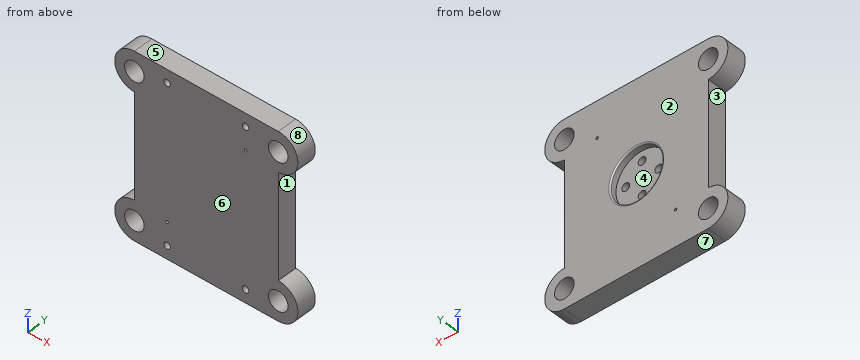
```python
from build123d import *

# Parameters (mm, degrees)
SKETCH1_R                                        = 15
BOSS_EXTRUDE1_DEPTH                              = 30
CBORE_FOR_M8_PAN_HEAD_MACHINE_SCREW1_D           = 9
CBORE_FOR_M8_PAN_HEAD_MACHINE_SCREW1_CBORE_D     = 18
CBORE_FOR_M8_PAN_HEAD_MACHINE_SCREW1_CBORE_DEPTH = 6
SKETCH_1_R                                       = 2
CUT_EXTRUDE1_DEPTH                               = 201.249843945
SKETCH_3_R                                       = 5
CUT_EXTRUDE3_DEPTH                               = 20
SKETCH_4_R                                       = 40
CUT_EXTRUDE4_DEPTH                               = 10
FILLET1_R                                        = 2
SKETCH5_R                                        = 6
CUT_EXTRUDE7_DEPTH                               = 15


with BuildPart() as part:
    # Sketch1 → Boss-Extrude1 (new body)
    with BuildSketch(Plane(origin=(0, 0, 0), x_dir=(1, 0, 0), z_dir=(0, 1, 0))):
        with BuildLine():
            Line((-110, -140), (80, -140))
            Line((80, -140), (80, 140))
            Line((80, 140), (-110, 140))
            ThreePointArc((-110, 140), (-140, 110), (-110, 80))
            Line((-110, 80), (-110, -80))
            ThreePointArc((-110, -80), (-140, -110), (-110, -140))
        make_face()
        with Locations(Location((-110, 110, 0), (0, 0, 270))):
            Circle(SKETCH1_R, mode=Mode.SUBTRACT)
        with Locations(Location((-110, -110, 0), (0, 0, 270))):
            Circle(SKETCH1_R, mode=Mode.SUBTRACT)
    boss_extrude1 = extrude(amount=BOSS_EXTRUDE1_DEPTH)

    # CBORE for M8 Pan Head Machine Screw1 (through all)
    with Locations(Plane(origin=(0, 30, 0), x_dir=(1, 0, 0), z_dir=(0, 1, 0))):
        with Locations((60, 120), (-60, 120), (-60, -120), (60, -120)):
            CounterBoreHole(CBORE_FOR_M8_PAN_HEAD_MACHINE_SCREW1_D / 2, CBORE_FOR_M8_PAN_HEAD_MACHINE_SCREW1_CBORE_D / 2, CBORE_FOR_M8_PAN_HEAD_MACHINE_SCREW1_CBORE_DEPTH)

    # Mirror1: Boss-Extrude1 across plane
    add(boss_extrude1.mirror(Plane(origin=(0, 0, 0), x_dir=(0, 0, 1), z_dir=(1, 0, 0))))

    # 草图1 → Cut-Extrude1 (cut, through all)
    with BuildSketch(Plane(origin=(0, 30, 0), x_dir=(1, 0, 0), z_dir=(0, 1, 0))):
        with Locations(Location((-60, 85, 0), (0, 0, 270))):
            Circle(SKETCH_1_R)
        with Locations(Location((60, -85, 0), (0, 0, 270))):
            Circle(SKETCH_1_R)
    extrude(amount=-CUT_EXTRUDE1_DEPTH, mode=Mode.SUBTRACT)

    # 草图3 → Cut-Extrude3 (cut)
    with BuildSketch(Plane.XZ):
        with Locations(Location((-60, 120, 0), (0, 0, 270))):
            Circle(SKETCH_3_R)
        with Locations(Location((60, 120, 0), (0, 0, 90))):
            Circle(SKETCH_3_R)
        with Locations(Location((60, -120, 0), (0, 0, 270))):
            Circle(SKETCH_3_R)
        with Locations(Location((-60, -120, 0), (0, 0, 90))):
            Circle(SKETCH_3_R)
    extrude(amount=-CUT_EXTRUDE3_DEPTH, mode=Mode.SUBTRACT)

    # 草图4 → Cut-Extrude4 (cut)
    with BuildSketch(Plane(origin=(0, 30, 0), x_dir=(1, 0, 0), z_dir=(0, 1, 0))):
        with Locations(Location((0, 0, 0), (0, 0, 270))):
            Circle(SKETCH_4_R)
    extrude(amount=-CUT_EXTRUDE4_DEPTH, mode=Mode.SUBTRACT)

    # Fillet1
    fillet1_edges = [part.edges().sort_by_distance(p)[0] for p in [
        (0, 30, -40),
    ]]
    fillet(fillet1_edges, radius=FILLET1_R)

    # Sketch5 → Cut-Extrude7 (cut)
    with BuildSketch(Plane(origin=(0, 20, 0), x_dir=(1, 0, 0), z_dir=(0, 1, 0))):
        with Locations(Location((0, 25, 0), (0, 0, 270))):
            Circle(SKETCH5_R)
        with Locations(Location((-25.4, 0, 0), (0, 0, 270))):
            Circle(SKETCH5_R)
        with Locations(Location((25, 0, 0), (0, 0, 270))):
            Circle(SKETCH5_R)
        with Locations(Location((0, -25, 0), (0, 0, 270))):
            Circle(SKETCH5_R)
    extrude(amount=-CUT_EXTRUDE7_DEPTH, mode=Mode.SUBTRACT)


solid = part.part
```
The listing builds one solid part. Answer for the finished solid, in the listing's coordinates (mm). Face numbers are marked on the shaded views. A direction names the side the tool comes from. Coordinates: 2 decimals unless noted, no trailing zeros. Loops run counter-clockwise (first coordinate to the right, second up) from the corner with the lowest first, then second, coordinate; pieces in that order, holes last. Notation, with made-up numbers: (14.25, 55) -> (44.25, 55) arc R18 ccw to (44.25, 70) -> close; hole circle Ø1 at (-18, 13). An arc over 180 degrees is marked (long way). Use one line per item in the form item = value. Start each with the question number.
Item 1: Consider L1, parallel to X at y = 16, z = 110; L2, parallel to X at y = 11.75, z = 0; L3, parallel to Z at x = -109.5, y = 25.75. Determine where each line is inside the solid, lowest interval first. Write a range as [from, to].
Item 2: A tool of negligible diameter and unlimited length cuts with its end or side. For the marked faces 1, 2, 3, 4 and 5, from which of +Z, -Z, +X, -X, +Y, -Y can it reach the whole face along a straight path? Write none if from no direction.
Item 3: The mould has two halves that part along Z. Classify the marked faces 6, 7 and 8: released by +Z, released by -Z, zero draft, split by the parting line, or undercut.
Item 4: The part is cut by section B-B on y = 10.5. Count the separate pieces of the cut face and the enclosed holes in it, then the cut area to 3 significant figures.
Item 5: The part is cut by section D-D on x = 0. Determine the outline of the cut face in (y, z).
Item 6: The part is cut by section A-A on z = -110. Determine the outline of the cut face in (x, y), then the cut area to 3 significant figures.
Item 7: The part is cut by section C-C on x = -117. Determine the outline of the cut face in (y, z).
Item 8: Flat-ended cylindrical pins translate along their axes: pin 1 Ø15.5 at (x, z) = (0, -25) entering from +Y; pin 2 Ø12 at (y, z) = (16.5, 98.5) entering from -X; pin 3 Ø3.5 at (x, z) = (2, -28) entering from +Y; pin 4 Ø2.5 at (x, z) = (60, 85) entering from -Y. Find the tip coordinate at first contact, or state that the pin passes through.
Answer key:
q1.L1 = [-140, -125], [-95, 95], [125, 140]
q1.L2 = [-110, -31.4], [-19.4, 19], [31, 110]
q1.L3 = [-140, -124.99], [-95.01, 95.01], [124.99, 140]
q2.face_1 = +X, +Y, -Y
q2.face_2 = +Z, -Z, +X, -X, +Y
q2.face_3 = -X, +Y, -Y
q2.face_4 = +Y
q2.face_5 = +Z, +X, -X, +Y, -Y
q3.face_6 = zero draft
q3.face_7 = released by -Z
q3.face_8 = undercut
q4.separate_pieces = 1
q4.enclosed_holes = 14
q4.area = 63,600 mm2
q5.outline = (0, -140) -> (30, -140) -> (30, -42) arc R2 ccw to (28, -40) -> (20, -40) -> (20, -31) -> (5, -31) -> (5, -19) -> (20, -19) -> (20, 19) -> (5, 19) -> (5, 31) -> (20, 31) -> (20, 40) -> (28, 40) arc R2 ccw to (30, 42) -> (30, 140) -> (0, 140) -> close
q6.outline = (-140, 0) -> (-125, 0) -> (-125, 30) -> (-140, 30) -> close; (-95, 0) -> (95, 0) -> (95, 30) -> (-95, 30) -> close; (125, 0) -> (140, 0) -> (140, 30) -> (125, 30) -> close
q6.area = 6,600 mm2
q7.outline = (0, -139.17) -> (30, -139.17) -> (30, -123.27) -> (0, -123.27) -> close; (0, -96.73) -> (30, -96.73) -> (30, -80.83) -> (0, -80.83) -> close; (0, 80.83) -> (30, 80.83) -> (30, 96.73) -> (0, 96.73) -> close; (0, 123.27) -> (30, 123.27) -> (30, 139.17) -> (0, 139.17) -> close
q8.pin_1 = 20
q8.pin_2 = -139.49
q8.pin_3 = 5
q8.pin_4 = through
